Build history of the part. All positions in model axes, mm. Give positions to 0.01 mm unless a question says otherwise; leave off trailing zeros. Loops run counter-clockwise (first coordinate to the right, second up) from the corner with the lowest first, then second, coordinate; pieces in that order, holes last. Notation, with made-up numbers: (72, 79) -> (116, 79) arc R33 ccw to (116, 117) -> close; hole circle Ø5 at (29.25, -13). An arc over 180 degrees is marked (long way). Answer as a JSON object with one key per item and string values. Group by question number.
Q1. Band-saw the part on D-D, the plane z = 20.5. Write the cut outline in (x, y), plus the area to 3 significant figures.
Q2. Band-saw the part on A-A, the plane y = 0. Write the cut outline in (x, z), plus the area to 3 significant figures.
Q3. Drop flat-ended pins along their axis: pin 1 (5 mm diameter, centred on y = -5, z = 18, fed in from +X); pin 2 (1 mm diameter, centred on x = 25.5, z = 30.5, fed in from -Y); pin 3 (6 mm diameter, centred on x = -20, y = -35, fed in from +Z); pin 4 (6 mm diameter, centred on y = -15, z = 30, fed in from +X). Give the stop position or say it passes through.
Q4. Band-saw the part on C-C, the plane z = 15.5. Write the cut outline in (x, y).
Q5. Band-saw the part on B-B, the plane x = 0. Write the cut outline in (y, z), plus the area to 3 significant figures.
Q6. Wall check: probe 1 along Z at (x, y) = (0, 31); probe 2 along Y at (x, z) = (-12, 14); probe 3 along X at (y, z) = (-4, 32). Give the ranges that are in metal, low to high. Write a range as from..to.
Q7. Two-plate mould, pull along Y, no slides. Class faces 1 (the cylindrical face through (12.69, -24.397, 16.762)), 2 (the conical face through (40.199, 12.659, 0.146)), 3 (the flat face through (9, -27, 0)): pulls with the +Y half, pulls with the -Y half, needs draft (parallel to the pull), parting line crosses it, or undercut.
from build123d import *

# Parameters (mm, degrees)
SKETCH1_R               = 45
SKETCH1_R_2             = 27.5
BOSS_EXTRUDE1_DEPTH     = 34
CUT_EXTRUDE1_DEPTH      = 73.15261603
CUT_EXTRUDE1_DEPTH_BACK = 73.15261603
SKETCH3_R               = 6.5
CHAMFER1_SIZE           = 5
CHAMFER2_SIZE           = 3


with BuildPart() as part:
    # Sketch1 → Boss-Extrude1 (new body)
    with BuildSketch(Plane.XY):
        Circle(SKETCH1_R)
        Circle(SKETCH1_R_2, mode=Mode.SUBTRACT)
    extrude(amount=BOSS_EXTRUDE1_DEPTH)

    # Sketch3 → Cut-Extrude1 (cut, two sides: drawn at the far end of the back side and taken through both)
    with BuildSketch(Plane(origin=(0, 0, 0), x_dir=(1, 0, 0), z_dir=(0, 1, 0)).offset(-CUT_EXTRUDE1_DEPTH_BACK)):
        with Locations(Location((0, -17, 0), (0, 0, 270))):
            Circle(SKETCH3_R)
    extrude(amount=CUT_EXTRUDE1_DEPTH + CUT_EXTRUDE1_DEPTH_BACK, mode=Mode.SUBTRACT)

    # Chamfer1
    chamfer1_edges = [part.edges().sort_by_distance(p)[0] for p in [
        (-45, 0, 34),
    ]]
    chamfer(chamfer1_edges, length=CHAMFER1_SIZE)

    # Chamfer2
    chamfer2_edges = [part.edges().sort_by_distance(p)[0] for p in [
        (-45, 0, 0),
    ]]
    chamfer(chamfer2_edges, length=CHAMFER2_SIZE)


solid = part.part
Worked answers:
{
 "1": {"outline": "(-5.48, -44.67) -> (-5.48, -26.95) arc R27.5 cw to (-5.48, 26.95) -> (-5.48, 44.67) arc R45 ccw to start; (5.48, -44.67) arc R45 ccw to (5.48, 44.67) -> (5.48, 26.95) arc R27.5 cw to (5.48, -26.95) -> close", "area": "3,600 mm2"},
 "2": {"outline": "(-45, 3) -> (-42, 0) -> (-27.5, 0) -> (-27.5, 34) -> (-40, 34) -> (-45, 29) -> close; (27.5, 0) -> (42, 0) -> (45, 3) -> (45, 29) -> (40, 34) -> (27.5, 34) -> close", "area": "1,160 mm2"},
 "3": {"pin 1": "x = 44.93", "pin 2": "y = -35.95", "pin 3": "z = 34", "pin 4": "x = 43.32"},
 "4": {"outline": "(-6.32, -44.55) -> (-6.32, -26.76) arc R27.5 cw to (-6.32, 26.76) -> (-6.32, 44.55) arc R45 ccw to start; (6.32, -44.55) arc R45 ccw to (6.32, 44.55) -> (6.32, 26.76) arc R27.5 cw to (6.32, -26.76) -> close"},
 "5": {"outline": "(-45, 3) -> (-42, 0) -> (-27.5, 0) -> (-27.5, 10.5) -> (-45, 10.5) -> close; (-45, 23.5) -> (-27.5, 23.5) -> (-27.5, 34) -> (-40, 34) -> (-45, 29) -> close; (27.5, 0) -> (42, 0) -> (45, 3) -> (45, 10.5) -> (27.5, 10.5) -> close; (27.5, 23.5) -> (45, 23.5) -> (45, 29) -> (40, 34) -> (27.5, 34) -> close", "area": "701 mm2"},
 "6": {"probe 1": "0..10.5, 23.5..34", "probe 2": "-43.37..-24.74, 24.74..43.37", "probe 3": "-41.81..-27.21, 27.21..41.81"},
 "7": {"face 1": "undercut", "face 2": "parting line crosses it", "face 3": "needs draft"}
}
